CAD build for the part. Positions are in the model's coordinates, mm. A direction names the side the tool comes from. Coordinates: 2 decimals unless noted, no trailing zeros. Order: outer loops, then holes, each group sorted by start corner. A loop starts at its lowest first (then second) coordinate and runs counter-clockwise, first axis right, second up. Notation, with made-up numbers: (-14, 26) - (9, 26) arc R16 ccw to (9, 52) - close; hole circle Ø7 at (81.5, 76.5). An arc over 180 degrees is marked (long way). Write each question's results on one line, items separated by ' | '. Start each with the question number.
Q1. Which spindle directions (+Z, -Z, +X, -X, +Y, -Y) get a long thin tool onto all of the face, cutting with end or side? Do faces 1 (the flat face through (0, 0, 0)), 2 (the cylindrical face through (20.745, 3.905, 0.867)). Say none if no direction does.
Q2. Band-saw the part on D-D, the plane y = -3.5. Write the cut outline in (x, z), then the cut area to 3 significant figures.
Q3. Band-saw the part on A-A, the plane z = 0. Write the cut outline in (x, y).
Q4. Pin check, flat tips, straight feed: P1, Ø2, axis at x = 30, z = -2, coming from the +Y side; P2, Ø4, axis at x = 15, y = -0.5, coming from the -Z side; P3, Ø1.5, axis at x = 12.5, y = -1.5, coming from the -Z side; P4, Ø9, axis at y = 0, z = 0.5, coming from the -X side. Stop position of each tip, or through.
Q5. Band-saw the part on C-C, the plane x = 36. Write the cut outline in (y, z).
Q6. Wall check: probe 1 along X at (y, z) = (2.25, -6.5); probe 2 along Z at (x, y) = (24, 1.75); probe 3 along Y at (x, z) = (11, -1). Give the ranges that are in metal, low to high.
```python
from build123d import *


with BuildPart() as part:
    # Sketch1 → Revolve1 (revolve)
    with BuildSketch(Plane.XY, mode=Mode.PRIVATE) as revolve1_sk:
        Polygon((0, 0), (0, 3), (3, 3), (3, 4), (38, 4), (38, 8), (40, 8), (40, 0), align=None)
    revolve(revolve1_sk.sketch.rotate(Axis((40, 0, 0), (-1, 0, 0)), 90), axis=Axis((40, 0, 0), (-1, 0, 0)))


solid = part.part
```
Results below:
1) face 1: +Z, -Z, -X, +Y, -Y | face 2: -X
2) outline: (3, -1.94) - (38, -1.94) - (38, -7.19) - (40, -7.19) - (40, 7.19) - (38, 7.19) - (38, 1.94) - (3, 1.94) - close | area: 164 mm²
3) outline: (0, -3) - (3, -3) - (3, -4) - (38, -4) - (38, -8) - (40, -8) - (40, 8) - (38, 8) - (38, 4) - (3, 4) - (3, 3) - (0, 3) - close
4) P1: stops at y = 3.87 | P2: stops at z = -4 | P3: stops at z = -3.93 | P4: stops at x = 0
5) outline: circle Ø8 at (0, 0)
6) probe 1: x = 38 to 40 | probe 2: z = -3.6 to 3.6 | probe 3: y = -3.87 to 3.87
